```python
from build123d import *

# Parameters (mm, degrees)
BOSS_EXTRUDE1_DEPTH                                  = 9.5
HOLE_SIZE_PER_SOCKET_HEAD_CAP_SCREW_TYPE_D           = 5.5
HOLE_SIZE_PER_SOCKET_HEAD_CAP_SCREW_TYPE_CBORE_D     = 10
HOLE_SIZE_PER_SOCKET_HEAD_CAP_SCREW_TYPE_CBORE_DEPTH = 5.7
SKETCH4_W                                            = 5.5
SKETCH4_H                                            = 10
CUT_EXTRUDE1_DEPTH                                   = 5.7
SKETCH5_W                                            = 30
SKETCH5_H                                            = 11
CUT_EXTRUDE2_DEPTH                                   = 10
CHAMFER1_SIZE                                        = 1
FILLET1_R                                            = 2


with BuildPart() as part:
    # Sketch1 → Boss-Extrude1 (new, symmetric)
    with BuildSketch(Plane.XY):
        Polygon((28, 0), (-28, 0), (-28, 10), (-15, 10), (-15, 20), (15, 20), (15, 10), (28, 10), align=None)
    extrude(amount=BOSS_EXTRUDE1_DEPTH, both=True)

    # Hole size per socket head cap screw type 1 (through all)
    with Locations(Plane(origin=(0, 10, 0), x_dir=(-1, 0, 0), z_dir=(0, 1, 0))):
        with Locations((22.5, 0), (-22.5, 0)):
            CounterBoreHole(HOLE_SIZE_PER_SOCKET_HEAD_CAP_SCREW_TYPE_D / 2, HOLE_SIZE_PER_SOCKET_HEAD_CAP_SCREW_TYPE_CBORE_D / 2, HOLE_SIZE_PER_SOCKET_HEAD_CAP_SCREW_TYPE_CBORE_DEPTH)

    # Sketch4 → Cut-Extrude1 (cut)
    with BuildSketch(Plane(origin=(0, 10, 0), x_dir=(1, 0, 0), z_dir=(0, 1, 0))):
        with Locations((-25.25, 0)):
            Rectangle(SKETCH4_W, SKETCH4_H)
        with Locations((25.25, 0)):
            Rectangle(SKETCH4_W, SKETCH4_H)
    extrude(amount=-CUT_EXTRUDE1_DEPTH, mode=Mode.SUBTRACT)

    # Sketch5 → Cut-Extrude2 (cut)
    with BuildSketch(Plane(origin=(0, 20, 0), x_dir=(1, 0, 0), z_dir=(0, 1, 0))):
        with Locations((0, 9.5)):
            Rectangle(SKETCH5_W, SKETCH5_H)
        with Locations((0, -9.5)):
            Rectangle(SKETCH5_W, SKETCH5_H)
    extrude(amount=-CUT_EXTRUDE2_DEPTH, mode=Mode.SUBTRACT)

    # Chamfer1
    chamfer1_edges = [part.edges().sort_by_distance(p)[0] for p in [
        (-28, 5, 9.5),
        (28, 5, 9.5),
        (28, 5, -9.5),
        (-28, 5, -9.5),
    ]]
    chamfer(chamfer1_edges, length=CHAMFER1_SIZE)

    # Fillet1
    fillet1_edges = [part.edges().sort_by_distance(p)[0] for p in [
        (-15, 20, 0),
        (15, 20, 0),
    ]]
    fillet(fillet1_edges, radius=FILLET1_R)


solid = part.part
```
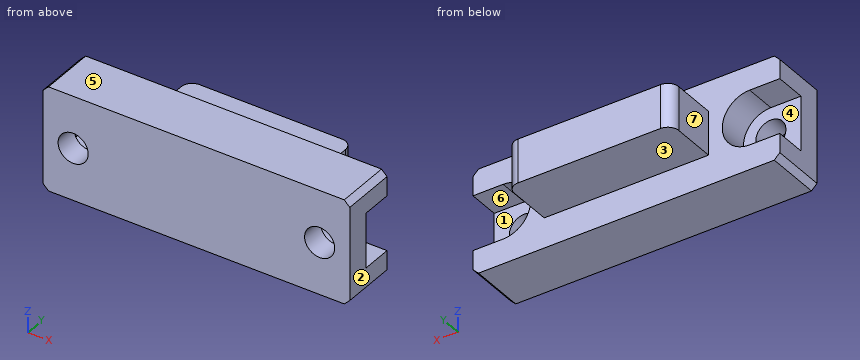
Could you check a few things on this model? Use its own coordinates, in mm. Face numbers are marked on the shaded views. A direction names the side the tool comes from. Round coordinates to 2 decimals unless told otherwise and drop trailing zeros. Write each loop counter-clockwise with the first axis right and the second up, starting at its lowest first coordinate (ties: lowest second). Pieces come first, ordered by that corner, then holes. Notation, with made-up numbers: M 17.5,15 L 58.5,15 A23 cw 58.5,34 Z; hole C 55,7 d7. An arc over 180 degrees is marked long. Answer in a Markdown table with one row per item. Add a question column.
Q1. Imagine slicing it at A-A (z = 0). Please give me the cut outline in (x, y).
Q2. Imagine slicing it at B-B (y = 1.5). Please give me the cut outline in (x, z), then the cut area to 3 significant figures.
Q3. On a 3-axis mill with a long thin cutter (end or side, diameter ignored), from which of +Z, -Z, +X, -X, +Y, -Y can I reach the whole of each face in a straight line? I mean the marked faces 4, 5, 6 and 7. Say none if no direction works.
Q4. Will these pins go through, and if not, where does the flat tip stop? pin 1 Ø5 at (x, y) = (-3.5, 13.5) entering from -Z; pin 2 Ø4 at (y, z) = (13.5, -2) entering from +X; pin 3 Ø1.5 at (x, y) = (6, 15.5) entering from +Z.
Q5. Imagine slicing it at C-C (x = -7.5). Please give me the cut outline in (y, z).
Q6. Imagine slicing it at D-D (z = 7). Please give me the cut outline in (x, y).
Q7. If we mould it in two halves opening along Z, with no side actions, what happens to the marked faces 1, 2 and 3? For each: +Z half, -Z half, draft (parallel to the pull), parting line (faces both ways), or undercut.
Q8. If I drill on line 1 (X direction, y = 2.9, z = 0); line 2 (Z direction, x = 22.5, y = 1.95); line 3 (X direction, y = 3.5, z = 1.25), over which ranges is the centre line in solid material (lowest first)? Write a range as from..to.
Values:
| question | item | result |
|---|---|---|
| 1 | outline | M -28,0 L -25.25,0 L -25.25,4.3 L -28,4.3 Z; M -19.75,0 L 19.75,0 L 19.75,4.3 L 17.5,4.3 L 17.5,10 L 15,10 L 15,18 A2 ccw 13,20 L -13,20 A2 ccw -15,18 L -15,10 L -17.5,10 L -17.5,4.3 L -19.75,4.3 Z; M 25.25,0 L 28,0 L 28,4.3 L 25.25,4.3 Z |
| 2 | outline | M -28,-8.5 L -27,-9.5 L 27,-9.5 L 28,-8.5 L 28,8.5 L 27,9.5 L -27,9.5 L -28,8.5 Z; hole C -22.5,0 d5.5; hole C 22.5,0 d5.5 |
| 2 | area | 1,010 mm^2 |
| 3 | face 4 | -X, +Y |
| 3 | face 5 | +Z, +X, -X, +Y, -Y |
| 3 | face 6 | +X, +Y |
| 3 | face 7 | +Z, -Z, -X, +Y |
| 4 | pin 1 | z = -4 |
| 4 | pin 2 | x = 15 |
| 4 | pin 3 | z = 4 |
| 5 | outline | M 0,-9.5 L 10,-9.5 L 10,-4 L 20,-4 L 20,4 L 10,4 L 10,9.5 L 0,9.5 Z |
| 6 | outline | M -28,0 L 28,0 L 28,10 L -28,10 Z |
| 7 | face 1 | undercut |
| 7 | face 2 | draft |
| 7 | face 3 | -Z half |
| 8 | line 1 | -28..-25.25, -19.75..19.75, 25.25..28 |
| 8 | line 2 | -9.5..-2.75, 2.75..9.5 |
| 8 | line 3 | -28..-24.95, -20.05..20.05, 24.95..28 |
